```python
from build123d import *

# Parameters (mm, degrees)
F_4_5_4_5_DIAMETER_HOLE1_D     = 4.5
F_4_5_4_5_DIAMETER_HOLE1_DEPTH = 18
F_4_5_4_5_DIAMETER_HOLE1_TIP   = 1.351936393
SKETCH4_OUTSIDE_W              = 91.864
SKETCH4_OUTSIDE_H              = 91.864
SKETCH4_OUTSIDE_W_2            = 83.56481814
SKETCH4_OUTSIDE_H_2            = 62
CUT_EXTRUDE1_DEPTH             = 51.139804547


with BuildPart() as part:
    # Sketch1 → Revolve1 (revolve)
    with BuildSketch(Plane.XY, mode=Mode.PRIVATE) as revolve1_sk:
        Polygon((17.5, 0), (35, 0), (35, 6), (25.5, 6), (25.5, 8), (21.5, 8), (21.5, 7), (20, 6), (17.5, 6), align=None)
    revolve(revolve1_sk.sketch.rotate(Axis((0, 112.43124941, 0), (0, -1, 0)), 90), axis=Axis((0, 112.43124941, 0), (0, -1, 0)))

    # Ø4.5 (4.5) Diameter Hole1
    with Locations(Plane(origin=(0, 0, 0), x_dir=(-1, 0, 0), z_dir=(0, -1, 0))):
        with Locations((-22.5, 20), (-22.5, -20), (22.5, 20), (22.5, -20)):
            Hole(F_4_5_4_5_DIAMETER_HOLE1_D / 2, depth=F_4_5_4_5_DIAMETER_HOLE1_DEPTH)
            with Locations((0, 0, -(F_4_5_4_5_DIAMETER_HOLE1_DEPTH + F_4_5_4_5_DIAMETER_HOLE1_TIP / 2))):  # 118° drill point
                Cone(0, F_4_5_4_5_DIAMETER_HOLE1_D / 2, F_4_5_4_5_DIAMETER_HOLE1_TIP, mode=Mode.SUBTRACT)

    # Sketch4 outside → Cut-Extrude1 (cut, through all)
    with BuildSketch(Plane.XZ):
        Rectangle(SKETCH4_OUTSIDE_W, SKETCH4_OUTSIDE_H)
        Rectangle(SKETCH4_OUTSIDE_W_2, SKETCH4_OUTSIDE_H_2, mode=Mode.SUBTRACT)
    extrude(amount=-CUT_EXTRUDE1_DEPTH, mode=Mode.SUBTRACT)


solid = part.part
```
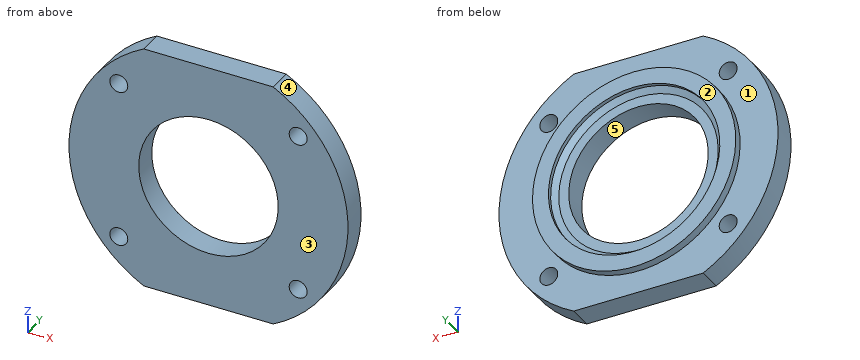
CAD build for the part. Positions are in the model's coordinates, mm. Face numbers are marked on the shaded views. A direction names the side the tool comes from. Round coordinates to 2 decimals unless told otherwise and drop trailing zeros. Order: outer loops, then holes, each group sorted by start corner. A loop starts at its lowest first (then second) coordinate and runs counter-clockwise, first axis right, second up. Notation, with made-up numbers: (44, -5) - (49, -5) arc R33 cw to (49, 26) - close; hole circle Ø8 at (74, 52). An arc over 180 degrees is marked (long way). Answer in a Markdown table with one row per item. Add a question column.
(1) Probe L1, parallel to Z at x = 22.5, y = 4.75; L2, parallel to X at y = 5.5, z = 0.5; L3, parallel to X at y = 2.8, z = -20. List the from-to ranges inside material, lowest first. Write a range as [from, to].
(2) Drop flat-ended pins along their axis: pin 1 Ø4 at (x, y) = (-21, 3.5) entering from +Z; pin 2 Ø3 at (y, z) = (4.5, -15.5) entering from +X; pin 3 Ø20 at (x, z) = (7, 6) entering from +Y. Give the stop position or say it passes through.
(3) Mould opens along X. For the marked faces 3, 4 and 5 say: +X half, -X half, draft (parallel to the pull), parting line (faces both ways), or undercut.
(4) Band-saw the part on D-D on x = 22.5. List the corners of the cut face in (y, z).
(5) Band-saw the part on B-B on x = 0. List the corners of the cut face in (y, z).
(6) Band-saw the part on A-A on z = 0. List the corners of the cut face in (x, y).
(7) Band-saw the part on C-C on y = 5. List the corners of the cut face in (x, z).
(8) 3-axis set-ups, long thin cutter, end or side, ignore diameter. For the marked faces 1 and 2: which of +Z, -Z, +X, -X, +Y, -Y reach the whole face in a straight line?
Data:
| question | item | result |
|---|---|---|
| 1 | L1 | z = [-26.81, -22.25], [-17.75, 17.75], [22.25, 26.81] |
| 1 | L2 | x = [-35, -17.49], [17.49, 35] |
| 1 | L3 | x = [-28.72, -24.75], [-20.25, 20.25], [24.75, 28.72] |
| 2 | pin 1 | stops at z = 29.39 |
| 2 | pin 2 | stops at x = 32.08 |
| 2 | pin 3 | stops at y = 6 |
| 3 | face 3 | draft |
| 3 | face 4 | +X half |
| 3 | face 5 | undercut |
| 4 | outline | (0, -26.81) - (6, -26.81) - (6, -22.25) - (0, -22.25) - close; (0, -17.75) - (6, -17.75) - (6, -12) - (8, -12) - (8, 12) - (6, 12) - (6, 17.75) - (0, 17.75) - close; (0, 22.25) - (6, 22.25) - (6, 26.81) - (0, 26.81) - close |
| 5 | outline | (0, -31) - (6, -31) - (6, -25.5) - (8, -25.5) - (8, -21.5) - (7, -21.5) - (6, -20) - (6, -17.5) - (0, -17.5) - close; (0, 17.5) - (6, 17.5) - (6, 20) - (7, 21.5) - (8, 21.5) - (8, 25.5) - (6, 25.5) - (6, 31) - (0, 31) - close |
| 6 | outline | (-35, 0) - (-17.5, 0) - (-17.5, 6) - (-20, 6) - (-21.5, 7) - (-21.5, 8) - (-25.5, 8) - (-25.5, 6) - (-35, 6) - close; (17.5, 0) - (35, 0) - (35, 6) - (25.5, 6) - (25.5, 8) - (21.5, 8) - (21.5, 7) - (20, 6) - (17.5, 6) - close |
| 7 | outline | (-16.25, -31) - (16.25, -31) arc R35 ccw to (16.25, 31) - (-16.25, 31) arc R35 ccw to start; hole circle Ø4.5 at (-22.5, -20); hole circle Ø4.5 at (-22.5, 20); hole circle Ø35 at (0, 0); hole circle Ø4.5 at (22.5, -20); hole circle Ø4.5 at (22.5, 20) |
| 8 | face 1 | +Y |
| 8 | face 2 | +Z, -Z, +X, -X, +Y |
